Source: three-view drawing plus pictorial views. Frame: mm from the lowest corner of the part. A direction names the side the tool comes from. Give positions to 0.01 mm unless a question says otherwise; leave off trailing zeros. Write each loop counter-clockwise with the first axis right and the second up, starting at its lowest first coordinate (ties: lowest second). Pieces come first, ordered by that corner, then holes. Notation, with made-up numbers: (62.25, -2) - (106.25, -2) arc R18 ccw to (106.25, 8) - close; hole circle Ø7 at (24, 19.5). An arc over 180 degrees is marked (long way). One line per question, with ' | ' between items. Start each with the question number.
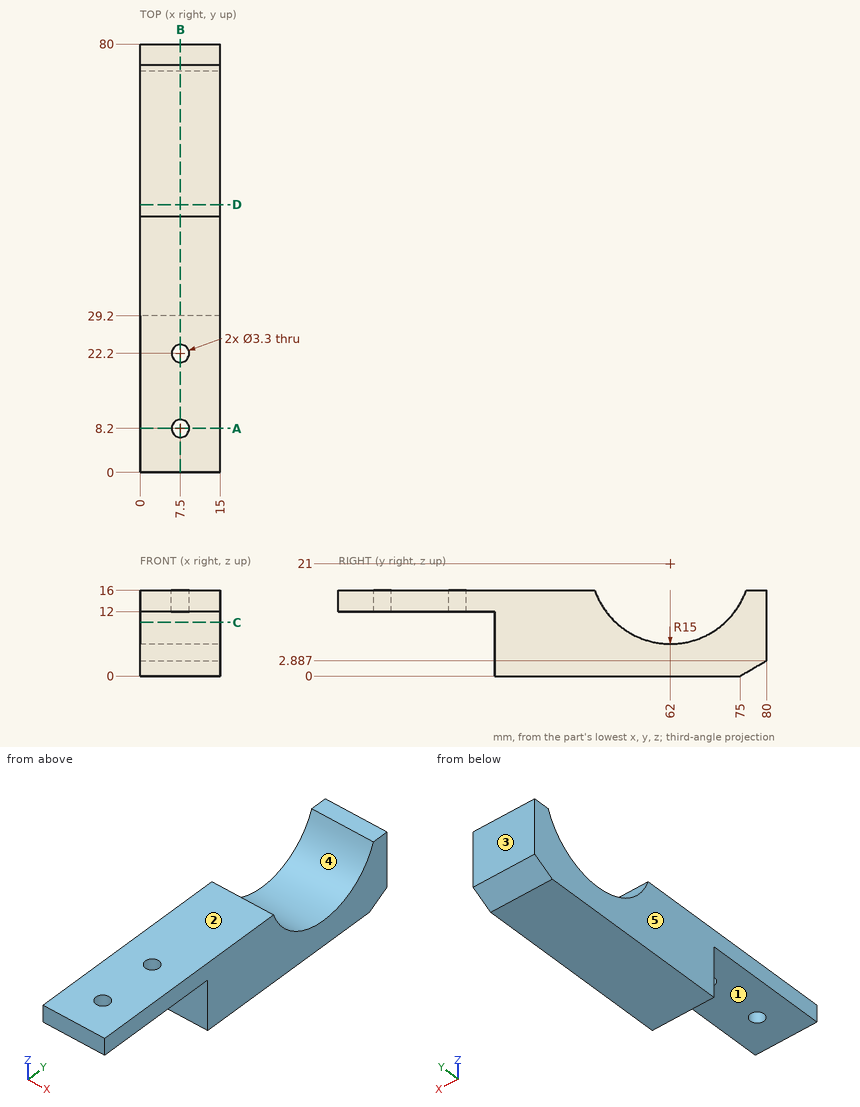
1) Section A-A, the plane y = 8.2. Output: boundary loops of the cut face in (x, z).
2) Pull-direction query (Y, two-part tool) for the marked faces 3, 4 and 5; classes: +Y half, -Y half, draft (parallel to the pull), parting line (faces both ways), or undercut.
3) Reachability of the marked faces 1 and 2 from +Z, -Z, +X, -X, +Y, -Y: full face, straight path, thin tool, end or side. Return the list, or none.
4) Line query: L1, parallel to Y at x = 7.5, z = 14.85; L2, parallel to Y at x = 7.5, z = 14; L3, parallel to Y at x = 4, z = 13. Output: solid intervals per line, ascending.
5) Section B-B, the plane x = 7.5. Output: boundary loops of the cut face in (y, z).
6) Section C-C, the plane z = 10. Output: boundary loops of the cut face in (x, y).
7) Section D-D, the plane y = 50. Output: boundary loops of the cut face in (x, z), plus the area to 3 significant figures.
8) First-contact query: pin 1 Ø4.5 at (x, y) = (9.5, 12) entering from -Z; pin 2 Ø8 at (x, y) = (8.5, 71) entering from +Z. Flat tips, straight axial feed; report the tip coordinate or a pass-through.
Answer key:
1) outline: (0, 12) - (5.85, 12) - (5.85, 16) - (0, 16) - close; (9.15, 12) - (15, 12) - (15, 16) - (9.15, 16) - close
2) face 3: +Y half | face 4: undercut | face 5: draft
3) face 1: -Z, +X, -X, -Y | face 2: +Z, +X, -X, +Y, -Y
4) L1: 0 to 6.55, 9.85 to 20.55, 23.85 to 48.32, 75.68 to 80 | L2: 0 to 6.55, 9.85 to 20.55, 23.85 to 48.73, 75.27 to 80 | L3: 0 to 49.31, 74.69 to 80
5) outline: (0, 12) - (6.55, 12) - (6.55, 16) - (0, 16) - close; (9.85, 12) - (20.55, 12) - (20.55, 16) - (9.85, 16) - close; (23.85, 12) - (29.2, 12) - (29.2, 0) - (75, 0) - (80, 2.89) - (80, 16) - (76.14, 16) arc R15 cw to (47.86, 16) - (23.85, 16) - close
6) outline: (0, 29.2) - (15, 29.2) - (15, 51.8) - (0, 51.8) - close; (0, 72.2) - (15, 72.2) - (15, 80) - (0, 80) - close
7) outline: (0, 0) - (15, 0) - (15, 12) - (0, 12) - close | area: 180 mm^2
8) pin 1: z = 12 | pin 2: z = 13.52
